from build123d import *

# Parameters (mm, degrees)
EXTRUDE_1_DEPTH      = 15
EXTRUDE_2_DEPTH      = 49.497475
EXTRUDE_2_DEPTH_BACK = 49.497475
CUT_EXTRUDE_3_DEPTH  = 113
SKETCH_8_R           = 3.3
CUT_EXTRUDE_4_DEPTH  = 113
CUT_EXTRUDE_START    = -15
SKETCH_9_R           = 6
CUT_EXTRUDE_5_DEPTH  = 113
CUT_EXTRUDE_6_DEPTH  = 25
SKETCH_11_R          = 2.2
CUT_EXTRUDE_7_DEPTH  = 30


with BuildPart() as part:
    # 草图1 → 凸台-拉伸1 (new, symmetric)
    with BuildSketch(Plane.XY):
        Polygon((0, 0), (70, 0), (0, -70), align=None)
    extrude(amount=EXTRUDE_1_DEPTH, both=True)

    # 草图5 → 凸台-拉伸2 (add, two sides: drawn at the far end of the back side and taken through both)
    with BuildSketch(Plane(origin=(0, 0, 0), x_dir=(0.7071067811865476, -0.7071067811865476, 0), z_dir=(-0.7071067811865476, -0.7071067811865476, 0)).offset(-EXTRUDE_2_DEPTH_BACK)):
        Polygon((65.854033042, -76.043506833), (49.497474683, -15), (38.68197258, -15), (55.763032203, -78.747382359), align=None)
    extrude(amount=EXTRUDE_2_DEPTH + EXTRUDE_2_DEPTH_BACK)

    # 草图7 → 切除-拉伸3 (cut)
    with BuildSketch(Plane.XY.offset(15)):
        Polygon((70, 0), (54.704570242, 0), (62.352285121, -7.647714879), align=None)
        Polygon((62.352285121, 7.647714879), (54.704570242, 0), (70, 0), align=None)
        Polygon((70, 0), (62.352285121, -7.647714879), (73.918118454, -19.213548212), (81.565833333, -11.565833333), align=None)
        Polygon((19.213548212, -73.918118454), (7.647714879, -62.352285121), (0, -70), (11.565833333, -81.565833333), align=None)
        Polygon((0, -70), (7.647714879, -62.352285121), (0, -54.704570242), align=None)
        Polygon((0, -70), (0, -54.704570242), (-7.647714879, -62.352285121), align=None)
    extrude(amount=-CUT_EXTRUDE_3_DEPTH, mode=Mode.SUBTRACT)

    # 草图8 → 切除-拉伸4 (cut)
    with BuildSketch(Plane(origin=(0, 0, 0), x_dir=(1, 0, 0), z_dir=(0, 1, 0))):
        with Locations(Location((34.704570242, 0, 0), (0, 0, 270))):
            Circle(SKETCH_8_R)
    cut_extrude_4 = extrude(amount=-CUT_EXTRUDE_4_DEPTH, mode=Mode.SUBTRACT)

    # 草图9 → 切除-拉伸5 (cut)
    with BuildSketch(Plane(origin=(0, 0, 0), x_dir=(1, 0, 0), z_dir=(0, 1, 0)).offset(CUT_EXTRUDE_START)):
        with Locations(Location((34.704570242, 0, 0), (0, 0, 270))):
            Circle(SKETCH_9_R)
    cut_extrude_5 = extrude(amount=-CUT_EXTRUDE_5_DEPTH, mode=Mode.SUBTRACT)

    # 草图10 → 切除-拉伸6 (cut)
    with BuildSketch(Plane.XY.offset(15)):
        Polygon((20, -20), (20, -50), (47.352285121, -22.647714879), (50, -20), align=None)
    extrude(amount=-CUT_EXTRUDE_6_DEPTH, mode=Mode.SUBTRACT)

    # 镜向2: 切除-拉伸4, 切除-拉伸5 across plane
    add(cut_extrude_4.mirror(Plane(origin=(0, 0, 0), x_dir=(0, 0, 1), z_dir=(-0.7071067811865476, -0.7071067811865476, 0))), mode=Mode.SUBTRACT)
    add(cut_extrude_5.mirror(Plane(origin=(0, 0, 0), x_dir=(0, 0, 1), z_dir=(-0.7071067811865476, -0.7071067811865476, 0))), mode=Mode.SUBTRACT)

    # 草图11 → 切除-拉伸7 (cut)
    with BuildSketch(Plane(origin=(30.003794137, -30.003794137, 11.369559199), x_dir=(0.18301270189221028, -0.18301270189221025, -0.9659258262890718), z_dir=(0.6830127018922219, -0.6830127018922217, 0.25881904510250797))):
        with Locations(Location((70.49666512, 33.68197258, 0), (0, 0, 90))):
            Circle(SKETCH_11_R)
        with Locations(Location((85.49666512, 33.68197258, 0), (0, 0, 90))):
            Circle(SKETCH_11_R)
        with Locations(Location((85.49666512, -33.68197258, 0), (0, 0, 90))):
            Circle(SKETCH_11_R)
        with Locations(Location((70.49666512, -33.68197258, 0), (0, 0, 90))):
            Circle(SKETCH_11_R)
    extrude(amount=-CUT_EXTRUDE_7_DEPTH, mode=Mode.SUBTRACT)


solid = part.part
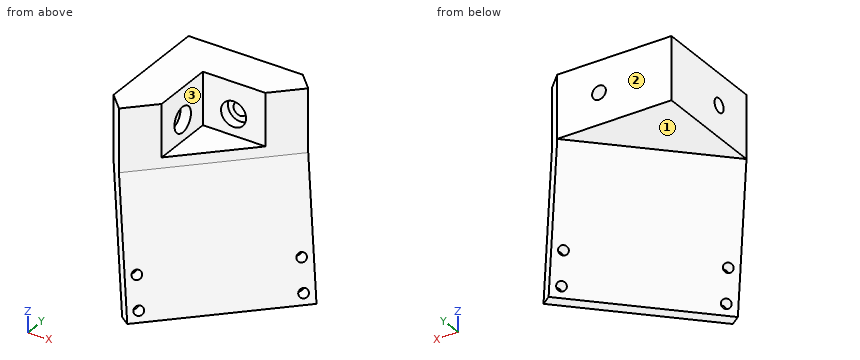
Check sheet for the modelled part. Datum: model origin and axes. Units: mm. Face numbers are marked on the shaded views. A direction names the side the tool comes from. Round coordinates to 2 decimals unless told otherwise and drop trailing zeros. Loops run counter-clockwise (first coordinate to the right, second up) from the corner with the lowest first, then second, coordinate; pieces in that order, holes last.
1. Set-up check for the marked faces 1, 2 and 3: record each of +Z, -Z, +X, -X, +Y, -Y from which the full face is reachable in a straight line by a thin tool's end or side.
2. Gauge pin test, flat ends, axial feed: pin 1 Ø12.5 at (y, z) = (-38, 6.5) entering from +X; pin 2 Ø4 at (x, z) = (34.7, 0) entering from -Y; pin 3 Ø6 at (x, z) = (62.5, -7.5) entering from -Y; pin 4 Ø1 at (y, z) = (-52, -67.5) entering from +X. Record the tip position at first contact, or that the pin passes through.
3. Sectioned sample at A-A on z = 0. Record the boundary of the cut face in (x, y), and give its area (3 significant figures).
4. Sectioned sample at C-C on z = -37.5. Record the boundary of the cut face in (x, y), and give its area (3 significant figures).
5. Sectioned sample at B-B on x = 46.5. Record the boundary of the cut face in (y, z).
6. Scan lines: probe 1 along X at (y, z) = (-12, 0); probe 2 along Y at (x, z) = (44, 1.5); probe 3 along X at (y, z) = (-16, 0). Record each from-to range of solid material in increasing order.
Recorded:
1. face 1: -Z, -X, +Y
1. face 2: +Z, -Z, +X, -X, +Y
1. face 3: +Z, +X, -Y
2. pin 1: stops at x = 20
2. pin 2: passes through
2. pin 3: stops at y = -10.5
2. pin 4: stops at x = 38.43
3. outline: (0, -54.7) - (7.65, -62.35) - (20, -50) - (20, -40.7) - (15, -40.7) - (15, -38) - (0, -38) - close; (0, -31.4) - (15, -31.4) - (15, -28.7) - (20, -28.7) - (20, -20) - (28.7, -20) - (28.7, -15) - (31.4, -15) - (31.4, 0) - (0, 0) - close; (38, -15) - (40.7, -15) - (40.7, -20) - (50, -20) - (62.35, -7.65) - (54.7, 0) - (38, 0) - close
3. area: 1,570 mm2
4. outline: (4.26, -58.97) - (11.91, -66.62) - (66.62, -11.91) - (58.97, -4.26) - close
4. area: 837 mm2
5. outline: (-46.63, -76.04) - (-32.36, -78.75) - (-8.2, -15) - (0, -15) - (0, 15) - (-20, 15) - (-20, -10) - (-23.5, -10) - (-23.5, -15) - close
6. probe 1: x = 0 to 31.4, 38 to 58
6. probe 2: y = -20 to 0
6. probe 3: x = 0 to 28.7, 40.7 to 54
